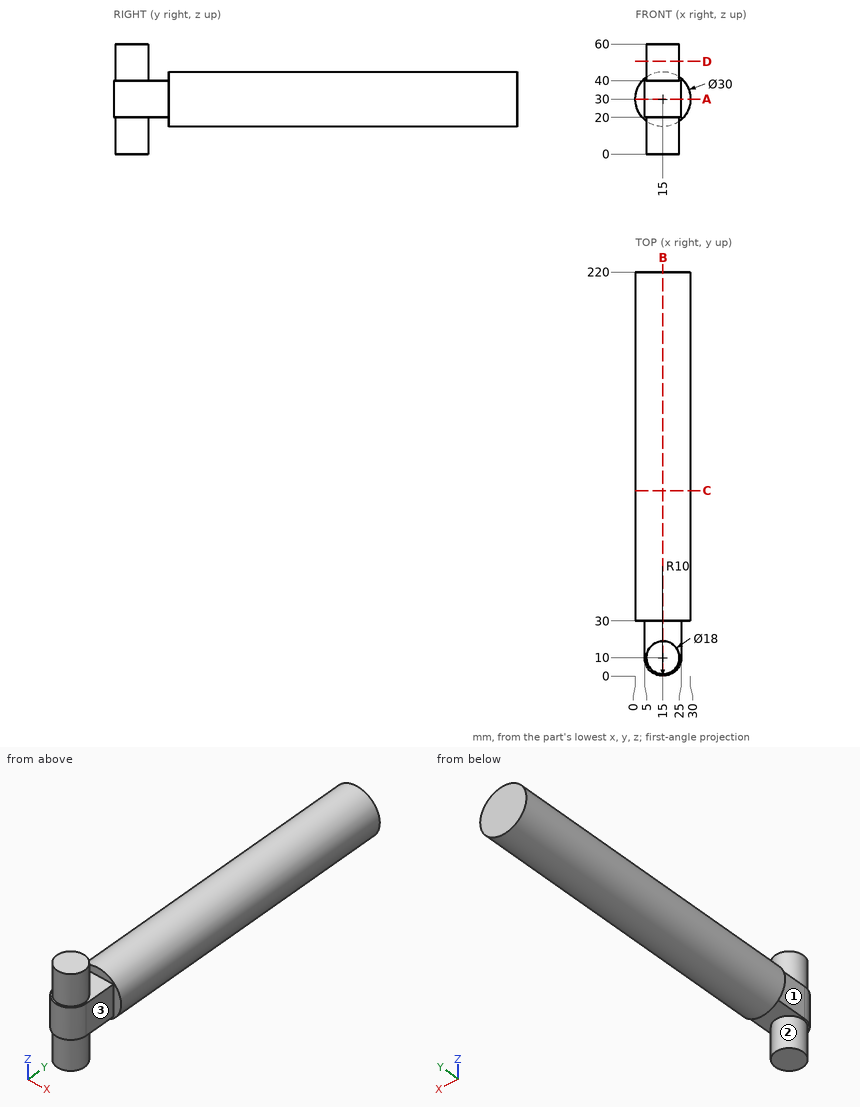
Part print with two shaded views. Sizes in mm from the minimum x, y, z corner. A direction names the side the tool comes from. Give positions to 0.01 mm unless a question says otherwise; leave off trailing zeros. Order: outer loops, then holes, each group sorted by start corner. A loop starts at its lowest first (then second) coordinate and runs counter-clockwise, first axis right, second up. Notation, with made-up numbers: M -28,-20 L -7,-20 A21 ccw -7,-12 Z; hole C 76.25,48.25 d1. An arc over 180 degrees is marked long. Put each result on its own line as item: value.
Item 1: Cut at B-B on x = 15. Write the cut outline in (y, z), then the cut area to 3 significant figures.
Results are:
outline: M 0,20 L 1,20 L 1,0 L 19,0 L 19,20 L 30,20 L 30,15 L 220,15 L 220,45 L 30,45 L 30,40 L 19,40 L 19,60 L 1,60 L 1,40 L 0,40 Z
area: 7,020 mm2
Item 2: Which spindle directions (+Z, -Z, +X, -X, +Y, -Y) get a long thin tool onto all of the face, cutting with end or side? Do the marked faces 1, 2 and 3. Say none if no direction does.
Results are:
face 1: +Z, -Z, -X, -Y
face 2: -Z
face 3: +Z, -Z, +X, -Y
Item 3: Cut at D-D on z = 50.5. Write the cut outline in (x, y), then the cut area to 3 significant figures.
Results are:
outline: C 15,10 d18
area: 254 mm2
Item 4: Cut at C-C on y = 101. Write the cut outline in (x, z), then the cut area to 3 significant figures.
Results are:
outline: C 15,30 d30
area: 707 mm2
Item 5: Wall check: probe 1 along Y at (x, z) = (14.75, 41); probe 2 along Z at (x, y) = (24.75, 11); probe 3 along Y at (x, z) = (26, 30). Give the ranges that are in metal, low to high.
Results are:
probe 1: 1 to 19, 30 to 220
probe 2: 20 to 40
probe 3: 30 to 220
Item 6: Drop flat-ended pins along their axis: pin 1 Ø4 at (x, z) = (27, 50.5) entering from +Y; pin 2 Ø12 at (y, z) = (61.5, 37.5) entering from -X; pin 3 Ø1 at (x, y) = (11.5, 46) entering from +Z; pin 4 Ø10 at (y, z) = (20, 34) entering from +X. Give the stop position or say it passes through.
Results are:
pin 1: through
pin 2: x = 0.08
pin 3: z = 44.7
pin 4: x = 25
Item 7: Cut at A-A on z = 30. Write the cut outline in (x, y), then the cut area to 3 significant figures.
Results are:
outline: M 0,30 L 5,30 L 5,10 A10 ccw 25,10 L 25,30 L 30,30 L 30,220 L 0,220 Z
area: 6,260 mm2
